For this review, take the finished solid that the model builds, in its own axes (mm). A direction names the side the tool comes from. Give positions to 0.01 mm unless a question says otherwise; leave off trailing zeros. Write each loop counter-clockwise with the first axis right and the second up, starting at its lowest first coordinate (ties: lowest second). Pieces come first, ordered by that corner, then holes.
Q1. Machinability: for faces 4 (the flat face through (150, -2, 0)), 5 (the flat face through (-2, 140, 0)), which of the approach directions +Z, -Z, +X, -X, +Y, -Y give a long, thin tool a straight path to every point of the face, cutting with its end or side? Answer none if there is none.
Q2. We need section B-B (y = 1.5). Write out the cut boundary in (x, z), then the cut area to 3 significant figures.
Q3. For line 1 (X direction, y = -89.5, z = -1.5), list the stretches that pass through material, from the lowest coordinate up.
Q4. Mouldability with a two-part tool opening along X and no side actions: class faces 1 (the flat face through (-150, -2, 0)), 2 (the flat face through (-2, 150, 0)), 3 (the flat face through (-140, -2, 0)) as released by +X, released by -X, zero draft, split by the parting line, or undercut.
Q5. We need section A-A (z = 1). Write out the cut boundary in (x, y), then the cut area to 3 significant figures.
```python
from build123d import *

# Parameters (mm, degrees)
SKETCH_1_W      = 300
SKETCH_1_H      = 300
SKETCH_1_W_2    = 280
SKETCH_1_H_2    = 280
EXTRUDE_1_DEPTH = 5


with BuildPart() as part:
    # 草图1 → 凸台-拉伸1 (new, symmetric)
    with BuildSketch(Plane.XY):
        Rectangle(SKETCH_1_W, SKETCH_1_H)
        Rectangle(SKETCH_1_W_2, SKETCH_1_H_2, mode=Mode.SUBTRACT)
    extrude(amount=EXTRUDE_1_DEPTH, both=True)


solid = part.part
```
Computed:
1. face 4: +Z, -Z, +X, +Y, -Y
1. face 5: +Z, -Z
2. outline: (-150, -5) - (-140, -5) - (-140, 5) - (-150, 5) - close; (140, -5) - (150, -5) - (150, 5) - (140, 5) - close
2. area: 200 mm2
3. line 1: x = -150 to -140, 140 to 150
4. face 1: released by -X
4. face 2: zero draft
4. face 3: undercut
5. outline: (-150, -150) - (150, -150) - (150, 150) - (-150, 150) - close; hole (-140, -140) - (140, -140) - (140, 140) - (-140, 140) - close
5. area: 11,600 mm2
